For this review, use the dimensioned drawing (mm, ordinates from the lowest corner) and the shaded views. Coordinates: 2 decimals unless noted, no trailing zeros. Loops run counter-clockwise (first coordinate to the right, second up) from the corner with the lowest first, then second, coordinate; pieces in that order, holes last. Notation, with made-up numbers: (70.5, 71) - (123.5, 71) arc R22 cw to (123.5, 85) - close; hole circle Ø5 at (89.5, 72.25). An arc over 180 degrees is marked (long way). Use a Markdown table: item, result. Add a question column.
1) Add section C-C, the plane y = 37. Give the boundary of the cut face in (x, z).
2) Add section A-A, the plane z = 4.25. Give the boundary of the cut face in (x, y), and give its area (3 significant figures).
3) Clearance check with flat-ended pins moving along their axes: pin 1 (6 mm diameter, centred on y = 7.5, z = 2, fed in from +X); pin 2 (4 mm diameter, centred on x = 34, z = 2, fed in from +Y). State where each tip first meets the part, or that it passes through.
4) To check wall thickness, follow L1, parallel to Y at x = 52, z = 5; L2, parallel to X at y = 8, z = 6.75; L3, parallel to Y at x = 28, z = 7. State the ranges of each line that lie inside material, in increasing order. Write a range as [from, to].
5) Add section B-B, the plane x = 51. Give the boundary of the cut face in (y, z).
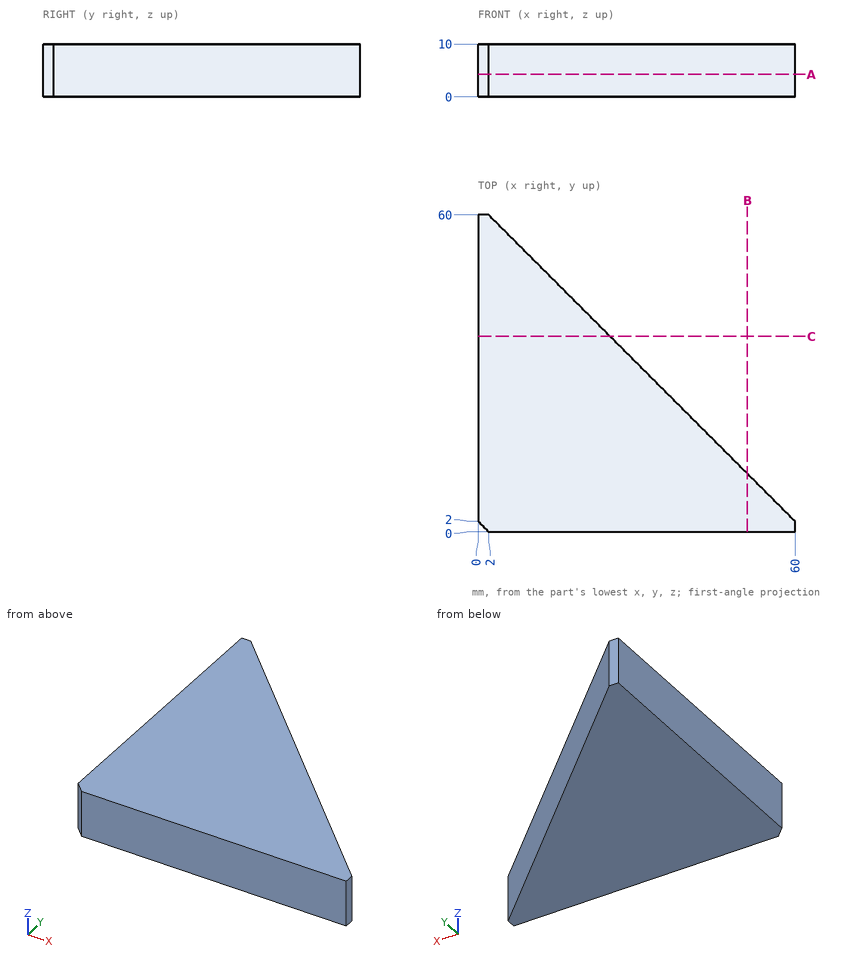
From the geometry:
| question | item | result |
|---|---|---|
| 1 | outline | (0, 0) - (25, 0) - (25, 10) - (0, 10) - close |
| 2 | outline | (0, 2) - (2, 0) - (60, 0) - (60, 2) - (2, 60) - (0, 60) - close |
| 2 | area | 1,920 mm^2 |
| 3 | pin 1 | stops at x = 57.5 |
| 3 | pin 2 | stops at y = 30 |
| 4 | L1 | y = [0, 10] |
| 4 | L2 | x = [0, 54] |
| 4 | L3 | y = [0, 34] |
| 5 | outline | (0, 0) - (11, 0) - (11, 10) - (0, 10) - close |
